```python
from build123d import *

# Parameters (mm, degrees)
SKETCH1_W                   = 600
SKETCH1_H                   = 700
BOSS_EXTRUDE1_DEPTH         = 9
FILLET1_R                   = 10
SKETCH3_R                   = 10
CUT_EXTRUDE2_DEPTH          = 41
SKETCH7_W                   = 8
SKETCH7_H                   = 12.747725193
CUT_EXTRUDE4_DEPTH          = 483.221865906
CUT_EXTRUDE8_START          = -499.177752008
SKETCH11_W                  = 6
SKETCH11_H                  = 19.989610894
SKETCH11_H_2                = 19.927609768
CUT_EXTRUDE8_DEPTH          = 881.951690015
LPATTERN4_COUNT             = 2
LPATTERN4_PITCH             = 379.75
LPATTERN5_COUNT             = 2
LPATTERN5_PITCH             = 450
LPATTERN5_START             = -499.177752008
LPATTERN5_COPY_1_SKETCH_W   = 6
LPATTERN5_COPY_1_SKETCH_H   = 19.989610894
LPATTERN5_COPY_1_SKETCH_H_2 = 19.927609768
LPATTERN5_COPY_1_DEPTH      = 881.951690015


with BuildPart() as part:
    # Sketch1 → Boss-Extrude1 (new body)
    with BuildSketch(Plane.XY):
        Rectangle(SKETCH1_W, SKETCH1_H)
    extrude(amount=BOSS_EXTRUDE1_DEPTH)

    # Fillet1
    fillet1_edges = [part.edges().sort_by_distance(p)[0] for p in [
        (300, -350, 4.5),
        (-300, -350, 4.5),
        (-300, 350, 4.5),
        (300, 350, 4.5),
    ]]
    fillet(fillet1_edges, radius=FILLET1_R)

    # Sketch3 → Cut-Extrude2 (cut)
    with BuildSketch(Plane(origin=(-23.01798078, 7.933390522, 0), x_dir=(-1, 0, 0), z_dir=(0, 0, -1))):
        with Locations((-208.01798078, 153.666609478)):
            Circle(SKETCH3_R)
        with Locations((-208.01798078, -216.333390522)):
            Circle(SKETCH3_R)
        with Locations((-208.01798078, -178.233390522)):
            Circle(SKETCH3_R)
        with Locations((173.98201922, 191.766609478)):
            Circle(SKETCH3_R)
        with Locations((173.98201922, 153.666609478)):
            Circle(SKETCH3_R)
        with Locations((173.98201922, -178.233390522)):
            Circle(SKETCH3_R)
        with Locations((173.98201922, -216.333390522)):
            Circle(SKETCH3_R)
        with Locations((-208.01798078, 191.766609478)):
            Circle(SKETCH3_R)
    extrude(amount=-CUT_EXTRUDE2_DEPTH, mode=Mode.SUBTRACT)

    # Sketch7 → Cut-Extrude4 (cut, through all)
    with BuildSketch(Plane(origin=(-23.01798078, 7.933390522, 0), x_dir=(-1, 0, 0), z_dir=(0, 0, -1))):
        with Locations((-246.01798078, -191.1057938)):
            Rectangle(SKETCH7_W, SKETCH7_H)
        with Locations((-246.01798078, -225.853518993)):
            Rectangle(SKETCH7_W, SKETCH7_H)
    extrude(amount=-CUT_EXTRUDE4_DEPTH, mode=Mode.SUBTRACT)

    # Sketch11 → Cut-Extrude8 (cut)
    with BuildSketch(Plane(origin=(-23.01798078, 7.93041319, -116.40444969), x_dir=(-1, 0, 0), z_dir=(1.1016286228319074e-14, -8.013698647454937e-05, -0.9999999967890317)).offset(CUT_EXTRUDE8_START)):
        with Locations((199.98201922, -115.795126315)):
            Rectangle(SKETCH11_W, SKETCH11_H)
        with Locations((199.98201922, -160.770464654)):
            Rectangle(SKETCH11_W, SKETCH11_H_2)
    cut_extrude8 = extrude(amount=CUT_EXTRUDE8_DEPTH, mode=Mode.SUBTRACT)

    # LPattern4: Cut-Extrude8 ×2
    with Locations(*[Vector(0, 0.9999999967890317, -8.013698647454937e-05) * (i * LPATTERN4_PITCH) for i in range(1, LPATTERN4_COUNT)]):
        add(cut_extrude8, mode=Mode.SUBTRACT)

    # LPattern5: Cut-Extrude8 ×2
    with Locations(*[(i * LPATTERN5_PITCH, 0, 0) for i in range(1, LPATTERN5_COUNT)]):
        add(cut_extrude8, mode=Mode.SUBTRACT)

    # LPattern5 copy 1 sketch → LPattern5 copy 1 (cut)
    with BuildSketch(Plane(origin=(426.98201922, 387.680411971, -116.434881711), x_dir=(-1, 0, 0), z_dir=(1.1016286228319074e-14, -8.013698647454937e-05, -0.9999999967890317)).offset(LPATTERN5_START)):
        with Locations((199.98201922, -115.795126315)):
            Rectangle(LPATTERN5_COPY_1_SKETCH_W, LPATTERN5_COPY_1_SKETCH_H)
        with Locations((199.98201922, -160.770464654)):
            Rectangle(LPATTERN5_COPY_1_SKETCH_W, LPATTERN5_COPY_1_SKETCH_H_2)
    extrude(amount=LPATTERN5_COPY_1_DEPTH, mode=Mode.SUBTRACT)


solid = part.part
```
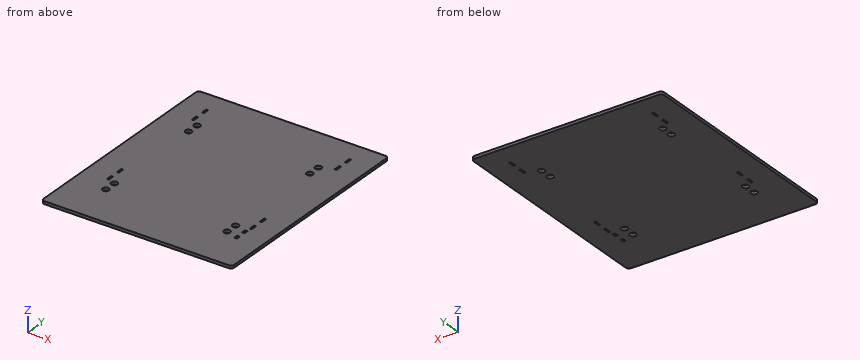
Model file for the job. Use its own axes, mm. Coordinates: 2 decimals unless noted, no trailing zeros. Order: outer loops, then holes, each group sorted by start corner. A loop starts at its lowest first (then second) coordinate and runs counter-clockwise, first axis right, second up. Notation, with made-up numbers: (68.25, 58.5) -> (77.25, 58.5) arc R27 cw to (77.25, 76.5) -> close; hole circle Ø11 at (-3, 11.5). An arc over 180 degrees is marked (long way). Answer as a JSON object with one key per item and string values. Group by question number.
1) Drill centre lines: L1, parallel to Y at x = -197, z = 5.75; L2, parallel to Y at x = 229, z = 2.75; L3, parallel to X at y = -167, z = 1. Where is each one in solid material? Low to high.
2) Cut at B-B, the plane x = -197. Write the cut outline in (y, z).
3) Cut at A-A, the plane y = 199.7. Write the cut outline in (x, z).
Check values:
{
 "1": {"L1": "y = -350 to -218.4, -198.4 to -180.3, -160.3 to 151.6, 171.6 to 189.7, 209.7 to 350", "L2": "y = -350 to -162.79, -142.87 to -117.85, -97.86 to 216.96, 236.88 to 261.9, 281.89 to 350", "L3": "x = -300 to -206.44, -187.56 to 175.56, 194.44 to 300"},
 "2": {"outline": "(-350, 0) -> (-218.4, 0) -> (-218.4, 9) -> (-350, 9) -> close; (-198.4, 0) -> (-180.3, 0) -> (-180.3, 9) -> (-198.4, 9) -> close; (-160.3, 0) -> (151.6, 0) -> (151.6, 9) -> (-160.3, 9) -> close; (171.6, 0) -> (189.7, 0) -> (189.7, 9) -> (171.6, 9) -> close; (209.7, 0) -> (350, 0) -> (350, 9) -> (209.7, 9) -> close"},
 "3": {"outline": "(-300, 0) -> (-207, 0) -> (-207, 9) -> (-300, 9) -> close; (-187, 0) -> (175, 0) -> (175, 9) -> (-187, 9) -> close; (195, 0) -> (300, 0) -> (300, 9) -> (195, 9) -> close"}
}
